```python
from build123d import *

# Parameters (mm, degrees)
BOSS_EXTRUDE1_START = -70
BOSS_EXTRUDE1_DEPTH = 70


with BuildPart() as part:
    # Sketch1 → Boss-Extrude1 (new body)
    with BuildSketch(Plane.XY.offset(BOSS_EXTRUDE1_START)):
        Polygon((90, 49), (84, 49), (84, 45), (90, 45), (90, 41.181900725), (88.106898586, 41.181900725), (88.106898586, 34.71973643), (69.860787635, 34.71973643), (69.860787635, -34.71973643), (88.106898586, -34.71973643), (88.106898586, -41.181900725), (90, -41.181900725), (90, -45), (84, -45), (84, -49), (90, -49), (90, -51.82740617), (81.240122505, -51.82740617), (81.240122505, -62.626229996), (-81.240122505, -62.626229996), (-81.240122505, -51.82740617), (-90, -51.82740617), (-90, -49), (-84, -49), (-84, -45), (-90, -45), (-90, -41.181900725), (-88.106898586, -41.181900725), (-88.106898586, -34.71973643), (-69.860787635, -34.71973643), (-69.860787635, 34.71973643), (-88.106898586, 34.71973643), (-88.106898586, 41.181900725), (-90, 41.181900725), (-90, 45), (-84, 45), (-84, 49), (-90, 49), (-90, 51.82740617), (-81.240122505, 51.82740617), (-81.240122505, 62.626229996), (81.240122505, 62.626229996), (81.240122505, 51.82740617), (90, 51.82740617), align=None)
        Polygon((65.860787635, -37.950818577), (65.860787635, 37.950818577), (85.261500452, 37.950818577), (85.261500452, 42.147480982), (81.240122505, 42.147480982), (81.240122505, 49), (77.240122505, 49), (77.240122505, 59.163837684), (-77.240122505, 59.163837684), (-77.240122505, 49), (-81.240122505, 49), (-81.240122505, 42.147480982), (-85.261500452, 42.147480982), (-85.261500452, 37.950818577), (-65.860787635, 37.950818577), (-65.860787635, -37.950818577), (-85.261500452, -37.950818577), (-85.261500452, -42.147480982), (-81.240122505, -42.147480982), (-81.240122505, -49), (-77.240122505, -49), (-77.240122505, -59.163837684), (77.240122505, -59.163837684), (77.240122505, -49), (81.240122505, -49), (81.240122505, -42.147480982), (85.261500452, -42.147480982), (85.261500452, -37.950818577), align=None, mode=Mode.SUBTRACT)
    extrude(amount=BOSS_EXTRUDE1_DEPTH)


solid = part.part
```
CAD build for the part. Positions are in the model's coordinates, mm. A direction names the side the tool comes from. Round coordinates to 2 decimals unless told otherwise and drop trailing zeros. Write each loop counter-clockwise with the first axis right and the second up, starting at its lowest first coordinate (ties: lowest second). Pieces come first, ordered by that corner, then holes.
Item 1: Tool access for faces 4 (the flat face through (-87, 49, -35)), 5 (the flat face through (86, 51.827, -35)), 6 (the flat face through (-85.262, 40, -35)): list every direction of +Z, -Z, +X, -X, +Y, -Y with a clear straight run to the whole face (end or side of a thin tool).
Filled in:
face 4: +Z, -Z, -X
face 5: +Z, -Z, +X, +Y
face 6: +Z, -Z
Item 2: Drop flat-ended pins along their axis: pin 1 Ø1.9 at (y, z) = (36.5, -23) entering from +X; pin 2 Ø1.5 at (x, z) = (89.5, -29) entering from -Y; pin 3 Ø1 at (y, z) = (8, -18) entering from +X. Give the stop position or say it passes through.
Filled in:
pin 1: stops at x = 88.11
pin 2: stops at y = -51.83
pin 3: stops at x = 69.86
Item 3: Mould opens along X. For faces 1 (the flat face through (1, -62.626, -35)), 2 (the flat face through (81.24, 57, -35)), 3 (the flat face through (-77.24, 54, -35)) say: released by +X, released by -X, zero draft, split by the parting line, or undercut.
Filled in:
face 1: zero draft
face 2: released by +X
face 3: undercut
Item 4: Band-saw the part on A-A on y = -54. Write the cut outline in (x, z).
Filled in:
outline: (-81.24, -70) - (-77.24, -70) - (-77.24, 0) - (-81.24, 0) - close; (77.24, -70) - (81.24, -70) - (81.24, 0) - (77.24, 0) - close
Item 5: Band-saw the part on B-B on x = -21.5. Write the cut outline in (y, z), then the cut area to 3 significant figures.
Filled in:
outline: (-62.63, -70) - (-59.16, -70) - (-59.16, 0) - (-62.63, 0) - close; (59.16, -70) - (62.63, -70) - (62.63, 0) - (59.16, 0) - close
area: 485 mm2
Item 6: Drill centre lines: L1, parallel to Y at x = -68, z = -59.5; L2, parallel to Y at x = 1, z = -57; L3, parallel to Y at x = 71, z = -42. Where is each one in solid material? Low to high.
Filled in:
L1: y = -62.63 to -59.16, -37.95 to 37.95, 59.16 to 62.63
L2: y = -62.63 to -59.16, 59.16 to 62.63
L3: y = -62.63 to -59.16, -37.95 to -34.72, 34.72 to 37.95, 59.16 to 62.63
